Can you work these out from the drawing? Everything is in mm from the part's minimum corner. Coordinates: 2 decimals unless noted, no trailing zeros. Loops run counter-clockwise (first coordinate to the right, second up) from the corner with the lowest first, then second, coordinate; pieces in that order, holes last. Notation, with made-up numbers: (9, 53) -> (34, 53) arc R8 ccw to (34, 66) -> close; hole circle Ø11 at (42, -4). An arc over 180 degrees is marked (long way). Put each result on its own line as item: value. Start each with the question number.
Item 1: Please list where these lines run through material, in increasing order: L1, parallel to Z at x = 193, y = 2 (1 decimal); L2, parallel to Z at x = 206, y = 10.5 (1 decimal); L3, parallel to X at y = 18.75, z = 50.5. Write a range as from..to.
Item 2: Will this pin go through, and if not, where does the flat tip stop? P1, Ø3, axis at x = 191.56, z = 41.56, coming from the +Y side.
Item 3: If we section it at A-A on z = 90: Please give me the cut outline in (x, y).
Item 4: If we section it at B-B on x = 150: Please give me the cut outline in (y, z), plus the area to 3 significant figures.
Item 5: If we section it at D-D on z = 37: Please give me the cut outline in (x, y), plus the area to 3 significant figures.
Item 6: If we section it at C-C on z = 55: Please give me the cut outline in (x, y).
Item 7: We'd pull the mould along X, two halves only. Please class the marked faces 1, 2 and 3: pulls with the +X half, pulls with the -X half, needs draft (parallel to the pull), parting line crosses it, or undercut.
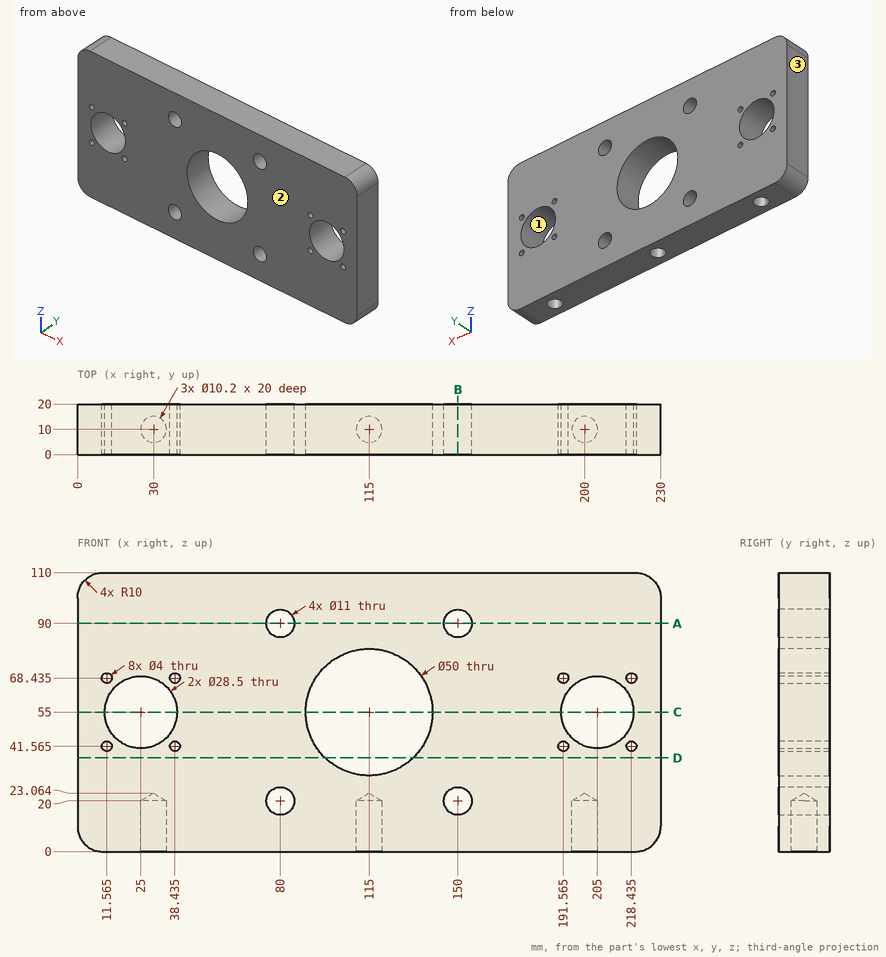
Solutions:
1. L1: 0..40.2, 43..47.3, 62.7..67, 69.8..110
1. L2: 0..40.8, 69.2..110
1. L3: 0..11.48, 38.52..90.41, 139.59..191.48, 218.52..230
2. P1: through
3. outline: (0, 0) -> (74.5, 0) -> (74.5, 20) -> (0, 20) -> close; (85.5, 0) -> (144.5, 0) -> (144.5, 20) -> (85.5, 20) -> close; (155.5, 0) -> (230, 0) -> (230, 20) -> (155.5, 20) -> close
4. outline: (0, 0) -> (20, 0) -> (20, 14.5) -> (0, 14.5) -> close; (0, 25.5) -> (20, 25.5) -> (20, 84.5) -> (0, 84.5) -> close; (0, 95.5) -> (20, 95.5) -> (20, 110) -> (0, 110) -> close
4. area: 1,760 mm^2
5. outline: (0, 0) -> (97.65, 0) -> (97.65, 20) -> (0, 20) -> close; (132.35, 0) -> (230, 0) -> (230, 20) -> (132.35, 20) -> close
5. area: 3,910 mm^2
6. outline: (0, 0) -> (10.75, 0) -> (10.75, 20) -> (0, 20) -> close; (39.25, 0) -> (90, 0) -> (90, 20) -> (39.25, 20) -> close; (140, 0) -> (190.75, 0) -> (190.75, 20) -> (140, 20) -> close; (219.25, 0) -> (230, 0) -> (230, 20) -> (219.25, 20) -> close
7. face 1: undercut
7. face 2: needs draft
7. face 3: pulls with the -X half
